Geometry check sheet. Reference: the model listing, model coordinates, mm. Round coordinates to 2 decimals unless told otherwise and drop trailing zeros. Loops run counter-clockwise (first coordinate to the right, second up) from the corner with the lowest first, then second, coordinate; pieces in that order, holes last. Notation, with made-up numbers: (-17.75, 28) -> (21.25, 28) arc R34 ccw to (21.25, 64) -> close; hole circle Ø10 at (-16, 36.25). An arc over 180 degrees is marked (long way). Use one line per item in the form item = value.
from build123d import *

# Parameters (mm, degrees)
SKETCH1_R           = 5.25
BOSS_EXTRUDE1_DEPTH = 8


with BuildPart() as part:
    # Sketch1 → Boss-Extrude1 (new body)
    with BuildSketch(Plane.XY):
        with BuildLine():
            Line((-32.5, 0), (32.5, 0))
            Line((32.5, 0), (8.762352479, 56.670310482))
            ThreePointArc((8.762352479, 56.670310482), (0, 62.5), (-8.762352479, 56.670310482))
            Line((-8.762352479, 56.670310482), (-32.5, 0))
        make_face()
        with Locations((0, 53)):
            Circle(SKETCH1_R, mode=Mode.SUBTRACT)
    extrude(amount=BOSS_EXTRUDE1_DEPTH)


solid = part.part
1. Gauge pin test, flat ends, axial feed: pin 1 (10 mm diameter, centred on x = -8, y = 10, fed in from -Z); pin 2 (1 mm diameter, centred on x = 9.5, z = 4, fed in from +Y); pin 3 (3 mm diameter, centred on y = 47.5, z = 5.5, fed in from -X); pin 4 (2 mm diameter, centred on y = 50, z = 1, fed in from -X). Record the tip position at first contact, or that the pin passes through.
Return value:
pin_1 = 0
pin_2 = 56.1
pin_3 = -13.23
pin_4 = -11.98
2. Section check B-B (z = 7). Record the boundary of the cut face in (x, y).
Return value:
outline = (-32.5, 0) -> (32.5, 0) -> (8.76, 56.67) arc R9.5 ccw to (-8.76, 56.67) -> close; hole circle Ø10.5 at (0, 53)
3. Section check C-C (x = -1.5). Record the boundary of the cut face in (y, z).
Return value:
outline = (0, 0) -> (47.97, 0) -> (47.97, 8) -> (0, 8) -> close; (58.03, 0) -> (62.38, 0) -> (62.38, 8) -> (58.03, 8) -> close
4. Mould release check, pull along Y, two halves, no side actions. Record for faces 1 (the cylindrical face through (4.85, 50.99, 3.94)), 2 (the flat face through (0, 0, 4)), 3 (the cylindrical face through (0.16, 62.5, 3.94)), 4 (the flat face through (0, 25, 8)): released by +Y, released by -Y, zero draft, split by the parting line, or undercut.
Return value:
face_1 = undercut
face_2 = released by -Y
face_3 = released by +Y
face_4 = zero draft
5. Material ranges on line 1 along Y through (x, z) = (0, 2.75); line 2 along Y through (x, z) = (4.5, 3.5); line 3 along X through (y, z) = (51, 6.25), recorded low to high.
Return value:
line_1 = 0 to 47.75, 58.25 to 62.5
line_2 = 0 to 50.3, 55.7 to 61.37
line_3 = -11.14 to -4.85, 4.85 to 11.14
6. Section check D-D (x = 10.5). Record the boundary of the cut face in (y, z).
Return value:
outline = (0, 0) -> (52.52, 0) -> (52.52, 8) -> (0, 8) -> close
7. Section check A-A (y = 49). Record the boundary of the cut face in (x, z), then the cut area to 3 significant figures.
Return value:
outline = (-11.98, 0) -> (-3.4, 0) -> (-3.4, 8) -> (-11.98, 8) -> close; (3.4, 0) -> (11.98, 0) -> (11.98, 8) -> (3.4, 8) -> close
area = 137 mm2
